from build123d import *

# Parameters (mm, degrees)
SKETCH_1_R      = 1.2
SKETCH_1_R_2    = 1.15
EXTRUDE_1_DEPTH = 0.8


with BuildPart() as part:
    # 草图1 → 凸台-拉伸1 (new body)
    with BuildSketch(Plane(origin=(0, 0, 0), x_dir=(1, 0, 0), z_dir=(0, 1, 0))):
        with BuildLine():
            Line((-1.079891697, 2.5), (2.931219678, 2.5))
            ThreePointArc((2.931219678, 2.5), (6.860663991, 0), (2.931219678, -2.5))
            Line((2.931219678, -2.5), (-1.079891697, -2.5))
            ThreePointArc((-1.079891697, -2.5), (-5.009336009, 0), (-1.079891697, 2.5))
        make_face()
        with Locations(Location((-2.249336009, 0, 0), (0, 0, 270))):
            Circle(SKETCH_1_R, mode=Mode.SUBTRACT)
        with Locations(Location((4.100663991, 0, 0), (0, 0, 270))):
            Circle(SKETCH_1_R_2, mode=Mode.SUBTRACT)
    extrude(amount=EXTRUDE_1_DEPTH)


solid = part.part
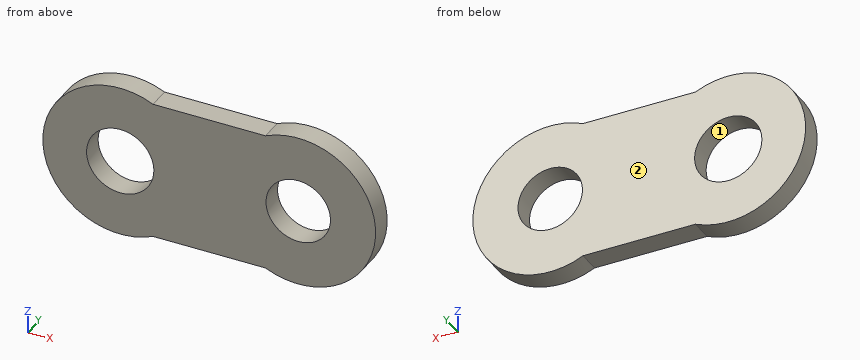
For this review, take the finished solid that the model builds, in its own axes (mm). Face numbers are marked on the shaded views. Give positions to 0.01 mm unless a question says otherwise; leave off trailing zeros. Order: outer loops, then holes, each group sorted by start corner. A loop starts at its lowest first (then second) coordinate and runs counter-clockwise, first axis right, second up. Notation, with made-up numbers: (26.5, 7.5) -> (34.5, 7.5) arc R24 cw to (34.5, 45.5) -> close; hole circle Ø10 at (-20, -6). An arc over 180 degrees is marked (long way). Write item = value, one per line.
1) We need section C-C, the plane y = 0.55. Give the boundary of the cut face in (x, z).
Findings:
outline = (-1.08, -2.5) -> (2.93, -2.5) arc R2.76 ccw (long way) to (2.93, 2.5) -> (-1.08, 2.5) arc R2.76 ccw (long way) to start; hole circle Ø2.4 at (-2.25, 0); hole circle Ø2.3 at (4.1, 0)
2) We need section A-A, the plane z = 0. Give the boundary of the cut face in (x, y).
Findings:
outline = (-5.01, 0) -> (-3.45, 0) -> (-3.45, 0.8) -> (-5.01, 0.8) -> close; (-1.05, 0) -> (2.95, 0) -> (2.95, 0.8) -> (-1.05, 0.8) -> close; (5.25, 0) -> (6.86, 0) -> (6.86, 0.8) -> (5.25, 0.8) -> close
3) Draft analysis for pull direction X (two halves, no side actions). For the marked faces 1 and 2, state which applies: pulls with the +X half, pulls with the -X half, needs draft (parallel to the pull), parting line crosses it, or undercut.
Findings:
face_1 = undercut
face_2 = needs draft
4) We need section D-D, the plane x = -0.75. Give the boundary of the cut face in (y, z), and give its area (3 significant figures).
Findings:
outline = (0, -2.5) -> (0.8, -2.5) -> (0.8, 2.5) -> (0, 2.5) -> close
area = 4.00 mm^2
5) We need section B-B, the plane x = 5. Give the boundary of the cut face in (y, z), and give its area (3 significant figures).
Findings:
outline = (0, -2.61) -> (0.8, -2.61) -> (0.8, -0.72) -> (0, -0.72) -> close; (0, 0.72) -> (0.8, 0.72) -> (0.8, 2.61) -> (0, 2.61) -> close
area = 3.03 mm^2
6) To check wall thickness, follow L1, parallel to X at y = 0.6, z = -0.4; L2, parallel to Z at x = 4.75, y = 0.4; L3, parallel to Z at x = -0.5, y = 0.55. State the ranges of each line that lie inside material, in increasing order. Write a range as from..to.
Findings:
L1 = -4.98..-3.38, -1.12..3.02, 5.18..6.83
L2 = -2.68..-0.95, 0.95..2.68
L3 = -2.5..2.5
